from build123d import *

# Parameters (mm, degrees)
BASE_BLOCK_SKETCH_W        = 85
BASE_BLOCK_SKETCH_H        = 60
BASE_BLOCK_85X60X16_DEPTH  = 16
UNDERSIDE_STEP_SKETCH_W    = 30
UNDERSIDE_STEP_SKETCH_H    = 4
UNDERSIDE_STEP_CUT_DEPTH   = 80.724525712
RELIEF_CUT_SKETCH_W        = 35
RELIEF_CUT_SKETCH_H        = 4
RELIEF_CUT_4MM_DEPTH       = 80.724525712
RAISED_BLOCK_20MM_DEPTH    = 20
TRIANGULAR_NOTCH_CUT_DEPTH = 5
HOLE_12_SKETCH_R           = 6
HOLE_12X10_DEPTH           = 10
FILLET_R2_R                = 2


with BuildPart() as part:
    # Base Block Sketch → Base Block 85x60x16 (new body)
    with BuildSketch(Plane(origin=(0, 0, 0), x_dir=(1, 0, 0), z_dir=(0, 1, 0))):
        with Locations((-7.5, 30)):
            Rectangle(BASE_BLOCK_SKETCH_W, BASE_BLOCK_SKETCH_H)
    extrude(amount=BASE_BLOCK_85X60X16_DEPTH)

    # Underside Step Sketch → Underside Step Cut (cut, through all)
    with BuildSketch(Plane.XY):
        with Locations((-35, 2)):
            Rectangle(UNDERSIDE_STEP_SKETCH_W, UNDERSIDE_STEP_SKETCH_H)
    extrude(amount=-UNDERSIDE_STEP_CUT_DEPTH, mode=Mode.SUBTRACT)

    # Relief Cut Sketch → Relief Cut 4mm (cut, through all)
    with BuildSketch(Plane.XY):
        with Locations((17.5, 2)):
            Rectangle(RELIEF_CUT_SKETCH_W, RELIEF_CUT_SKETCH_H)
    extrude(amount=-RELIEF_CUT_4MM_DEPTH, mode=Mode.SUBTRACT)

    # Raised Block Sketch → Raised Block 20mm (add)
    with BuildSketch(Plane(origin=(0, 16, 0), x_dir=(1, 0, 0), z_dir=(0, 1, 0))):
        Polygon((35, 60), (-15, 60), (-15, 50), (28, 0), (35, 0), align=None)
    extrude(amount=RAISED_BLOCK_20MM_DEPTH)

    # Notch Sketch → Triangular Notch Cut (cut)
    with BuildSketch(Plane(origin=(0, 16, 0), x_dir=(1, 0, 0), z_dir=(0, 1, 0))):
        Polygon((-25, 0), (-50, 25), (-50, 0), align=None)
    extrude(amount=-TRIANGULAR_NOTCH_CUT_DEPTH, mode=Mode.SUBTRACT)

    # Hole Ø12 Sketch → Hole Ø12x10 (cut)
    with BuildSketch(Plane(origin=(0, 16, 0), x_dir=(1, 0, 0), z_dir=(0, 1, 0))):
        with Locations(Location((-10, 20, 0), (0, 0, 270))):
            Circle(HOLE_12_SKETCH_R)
    extrude(amount=-HOLE_12X10_DEPTH, mode=Mode.SUBTRACT)

    # Fillet R2
    fillet_r2_edges = [part.edges().sort_by_distance(p)[0] for p in [
        (-10, 6, -26),
    ]]
    fillet(fillet_r2_edges, radius=FILLET_R2_R)


solid = part.part
The model under review builds one solid part; all positions refer to its coordinate system, in mm. A direction names the side the tool comes from. Coordinates: 2 decimals unless noted, no trailing zeros. Write each loop counter-clockwise with the first axis right and the second up, starting at its lowest first coordinate (ties: lowest second). Pieces come first, ordered by that corner, then holes. Notation, with made-up numbers: (29.5, -21) - (42.5, -21) arc R14 ccw to (42.5, -14) - close; hole circle Ø10 at (78.25, 18.25). An arc over 180 degrees is marked (long way). Answer as a JSON object with one key per item and string values. Group by question number.
1. Add section A-A (z = -42). Give the boundary of the cut face in (x, y).
2. To check wall thickness, follow probe 1 along X at (y, z) = (10, -20); probe 2 along Y at (x, z) = (19, -46); probe 3 along Y at (x, z) = (9.5, -2.5). State the ranges of each line that lie inside material, in increasing order.
3. Clearance check with flat-ended pins moving along their axes: pin 1 Ø4 at (x, z) = (-14, -7.5) entering from +Y; pin 2 Ø6.5 at (x, z) = (-9, -22) entering from +Y; pin 3 Ø1.2 at (y, z) = (2.5, -33.5) entering from -X. State where each tip first meets the part, or that it passes through.
4. Add section D-D (y = 25). Give the boundary of the cut face in (x, z), plus the area to 4 significant figures.
5. Mouldability with a two-part tool opening along X and no side actions: class faces 1 (the face through (-37, 14, -12)), 2 (the face through (-10, 0, -30)), 3 (the face through (35, 20, -30)), 4 (the face through (-13.65, 12.06, -24.76)) as pulls with the +X half, pulls with the -X half, needs draft (parallel to the pull), parting line crosses it, or undercut.
6. Add section C-C (x = -40.5). Give the boundary of the cut face in (y, z).
7. Add section B-B (y = 15). Give the boundary of the cut face in (x, z), plus the area to 3 significant figures.
8. Machinability: for faces 5 (the face through (-35, 4, -30)), 6 (the face through (-43, 11, -7)), 7 (the face through (-15, 26, -55)), 8 (the face through (0, 2, -30)), 9 (the face through (-10, 6, -20)), which of the approach directions +Z, -Z, +X, -X, +Y, -Y give a long, thin tool a straight path to every point of the face, cutting with its end or side? Answer none if there is none.
Findings:
{
 "1": {"outline": "(-50, 4) - (-20, 4) - (-20, 0) - (0, 0) - (0, 4) - (35, 4) - (35, 36) - (-8.12, 36) - (-8.12, 16) - (-50, 16) - close"},
 "2": {"probe 1": "-50 to -16, -4 to 35", "probe 2": "4 to 36", "probe 3": "4 to 16"},
 "3": {"pin 1": "y = 16", "pin 2": "y = 6.66", "pin 3": "x = -20"},
 "4": {"outline": "(-15, -60) - (35, -60) - (35, 0) - (28, 0) - (-15, -50) - close", "area": "1,925 mm²"},
 "5": {"face 1": "pulls with the -X half", "face 2": "needs draft", "face 3": "pulls with the +X half", "face 4": "undercut"},
 "6": {"outline": "(4, -60) - (16, -60) - (16, -15.5) - (11, -15.5) - (11, 0) - (4, 0) - close"},
 "7": {"outline": "(-50, -60) - (35, -60) - (35, 0) - (-25, 0) - (-50, -25) - close; hole circle Ø12 at (-10, -20)", "area": "4,670 mm²"},
 "8": {"face 5": "+Z, -Z, -X, -Y", "face 6": "+Z, -X, +Y", "face 7": "+Z, -Z, -X, +Y", "face 8": "+Z, -Z, +X, -Y", "face 9": "+Y"}
}
